```python
from build123d import *

# Parameters (mm, degrees)
SKETCH1_R           = 3
BOSS_EXTRUDE2_DEPTH = 1


with BuildPart() as part:
    # Sketch1 → Boss-Extrude2 (new body)
    with BuildSketch(Plane.XY):
        with BuildLine():
            Line((-23.148022373, -8.730243593), (-30.122846489, 12.649248922))
            ThreePointArc((-30.122846489, 12.649248922), (-29.288419203, 20.729586307), (-22.731208407, 25.524490657))
            ThreePointArc((-22.731208407, 25.524490657), (6.577970793, 27.774560597), (35.408236715, 22.038136022))
            ThreePointArc((35.408236715, 22.038136022), (41.345462771, 16.493997865), (41.208301592, 8.371848645))
            Line((41.208301592, 8.371848645), (31.728586192, -12.020940954))
            ThreePointArc((31.728586192, -12.020940954), (22.672300426, -8.599141601), (13.293379688, -6.198960674))
            ThreePointArc((13.293379688, -6.198960674), (11.656131568, -6.635918882), (10.941917146, -8.172607413))
            Line((10.941917146, -8.172607413), (10.944342154, -9.189079799))
            ThreePointArc((10.944342154, -9.189079799), (11.410804247, -10.468161557), (12.587919364, -11.152293875))
            ThreePointArc((12.587919364, -11.152293875), (13.423205338, -11.308812996), (14.256529596, -11.475461055))
            ThreePointArc((14.256529596, -11.475461055), (17.525943772, -13.786871862), (18.050961494, -17.7562604))
            Line((18.050961494, -17.7562604), (16.711120416, -22.40789263))
            ThreePointArc((16.711120416, -22.40789263), (15.785830822, -23.588348839), (14.300058147, -23.793573714))
            ThreePointArc((14.300058147, -23.793573714), (0.113320945, -22.031785702), (-14.073416257, -23.793573714))
            ThreePointArc((-14.073416257, -23.793573714), (-15.559188932, -23.588348839), (-16.484478526, -22.40789263))
            Line((-16.484478526, -22.40789263), (-17.824319603, -17.7562604))
            ThreePointArc((-17.824319603, -17.7562604), (-17.299301882, -13.786871862), (-14.029887705, -11.475461055))
            ThreePointArc((-14.029887705, -11.475461055), (-13.278530318, -11.324738612), (-12.525567944, -11.182250571))
            ThreePointArc((-12.525567944, -11.182250571), (-11.350088312, -10.495311954), (-10.886679055, -9.215120996))
            Line((-10.886679055, -9.215120996), (-10.886679055, -8.198645717))
            ThreePointArc((-10.886679055, -8.198645717), (-11.604557525, -6.663665462), (-13.242843438, -6.230614485))
            ThreePointArc((-13.242843438, -6.230614485), (-18.238041511, -7.311585647), (-23.148022373, -8.730243593))
        make_face()
        with Locations((12.060510133, -18.174977907)):
            Circle(SKETCH1_R, mode=Mode.SUBTRACT)
        with Locations((-11.981406179, -18.203656377)):
            Circle(SKETCH1_R, mode=Mode.SUBTRACT)
        with Locations((0, 14.968146711)):
            Circle(SKETCH1_R, mode=Mode.SUBTRACT)
        with Locations((24.591653109, 11.76043213)):
            Circle(SKETCH1_R, mode=Mode.SUBTRACT)
    extrude(amount=BOSS_EXTRUDE2_DEPTH)


solid = part.part
```
Here's how the part is built. I have some questions about the finished solid (model axes, mm). A direction names the side the tool comes from. Give positions to 0.01 mm unless a question says otherwise; leave off trailing zeros. Write each loop counter-clockwise with the first axis right and the second up, starting at its lowest first coordinate (ties: lowest second). Pieces come first, ordered by that corner, then holes. Notation, with made-up numbers: M 51,-33 L 61,-33 A7 cw 61,-23 Z; hole C 10.5,0 d4. An arc over 180 degrees is marked long. Put each result on its own line as item: value. Start each with the question number.
Item 1: If we section it at A-A, the plane y = 14: Write out the boundary of the cut face in (x, z).
Item 2: On a 3-axis mill with a long thin cutter (end or side, diameter ignored), from which of +Z, -Z, +X, -X, +Y, -Y can I reach the whole of each face in a straight line? I mean faces 1 (the cylindrical face through (-11.586, -6.679, 0.493)), 2 (the cylindrical face through (-11.36, -10.51, 0.49)), 3 (the flat face through (36.535, -1.682, 0.493)). Say none if no direction works.
Item 3: Thinking about a two-plate mould opening in Y: for faces 4 (the flat face through (-26.587, 1.81, 0.493)), 5 (the cylindrical face through (-18.2, -7.3, 0.5)), 6 (the flat face through (6, 8, 0)), which applies, +Y half, -Y half, draft (parallel to the pull), parting line (faces both ways), or undercut?
Item 4: If we section it at C-C, the plane z = 0.15: Write out the boundary of the cut face in (x, y).
Item 5: If we section it at D-D, the plane y = -17: Write out the boundary of the cut face in (x, z).
Item 6: If we section it at B-B, the plane x = 26: Write out the boundary of the cut face in (y, z), then the cut area to 3 significant figures.
Item 7: I need wall thicknesses on L1, parallel to Y at x = 0, z = 0.2; L2, parallel to Y at x = -14, z = 0.8; L3, parallel to X at y = 16.5, z = 0.55. Which ranges of each line are inside material? Lowest first, please. Write a range as from..to.
Values:
1. outline: M -30.46,0 L -2.84,0 L -2.84,1 L -30.46,1 Z; M 2.84,0 L 22.6,0 L 22.6,1 L 2.84,1 Z; M 26.59,0 L 42.04,0 L 42.04,1 L 26.59,1 Z
2. face 1: +Z, -Z
2. face 2: +Z, -Z, -X
2. face 3: +Z, -Z, +X, -Y
3. face 4: -Y half
3. face 5: undercut
3. face 6: draft
4. outline: M -30.12,12.65 L -23.15,-8.73 A75 cw -13.24,-6.23 A2 cw -10.89,-8.2 L -10.89,-9.22 A2 cw -12.53,-11.18 A70 ccw -14.03,-11.48 A5 ccw -17.82,-17.76 L -16.48,-22.41 A2 ccw -14.07,-23.79 A58 cw 14.3,-23.79 A2 ccw 16.71,-22.41 L 18.05,-17.76 A5 ccw 14.26,-11.48 A70 ccw 12.59,-11.15 A2 cw 10.94,-9.19 L 10.94,-8.17 A2 cw 13.29,-6.2 A87.48 cw 31.73,-12.02 L 41.21,8.37 A10 ccw 35.41,22.04 A108 ccw -22.73,25.52 A10 ccw Z; hole C -11.98,-18.2 d6; hole C 0,14.97 d6; hole C 12.06,-18.17 d6; hole C 24.59,11.76 d6
5. outline: M -17.98,0 L -14.73,0 L -14.73,1 L -17.98,1 Z; M -9.23,0 L 9.3,0 L 9.3,1 L -9.23,1 Z; M 14.82,0 L 18.21,0 L 18.21,1 L 14.82,1 Z
6. outline: M -9.72,0 L 9.11,0 L 9.11,1 L -9.72,1 Z; M 14.41,0 L 24.82,0 L 24.82,1 L 14.41,1 Z
6. area: 29.2 mm²
7. L1: -22.03..11.97, 17.97..27.97
7. L2: -23.78..-20.42, -15.98..-11.47, -6.37..27.04
7. L3: -30.59..-2.58, 2.58..41.34
